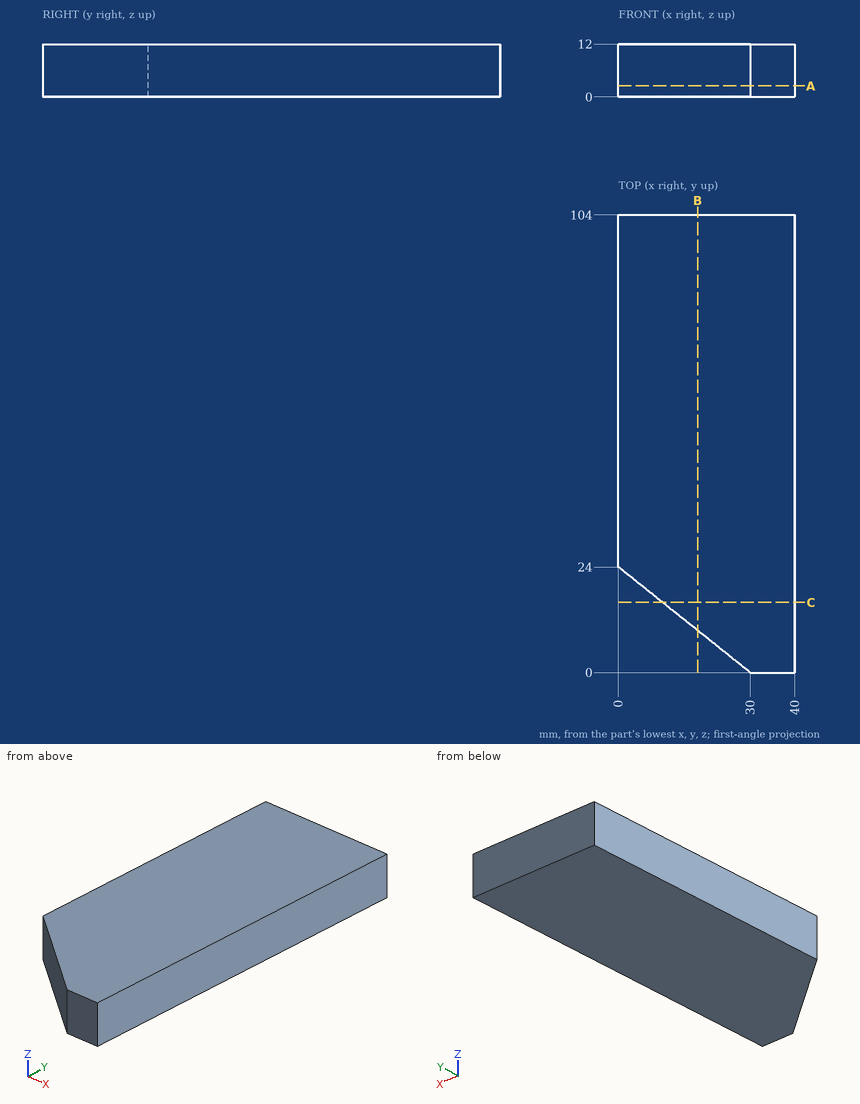
The drawing under review shows one solid part. Ordinate dimensions are in mm from its lowest x, y, z. Round coordinates to 2 decimals unless told otherwise and drop trailing zeros. Write each loop counter-clockwise with the first axis right and the second up, starting at its lowest first coordinate (ties: lowest second). Pieces come first, ordered by that corner, then holes.
(1) We need section C-C on y = 16. Give the boundary of the cut face in (x, z), and give its area (3 significant figures).
(2) Insertion check: pin 1 (2 mm diameter, centred on y = 19, z = 5.5, fed in from -X); pin 2 (2 mm diameter, centred on x = 9.5, z = 7.5, fed in from -Y); pin 3 (6 mm diameter, centred on x = 9, z = 1.5, fed in from -Y). Each pin has a flat end and moves straight along its axis. Give the tip position at first contact, or say it passes through.
(3) We need section A-A on z = 2.5. Give the boundary of the cut face in (x, y), and give its area (3 significant figures).
(4) We need section B-B on x = 18. Give the boundary of the cut face in (y, z).
(5) Wall thickness on L1, parallel to X at y = 12, z = 3; L2, parallel to Y at x = 29, z = 1.25; L3, parallel to Y at x = 27, z = 10.5: over which ranges is each line inside the solid? List them lowest first.
Findings below:
1. outline: (10, 0) - (40, 0) - (40, 12) - (10, 12) - close
1. area: 360 mm2
2. pin 1: stops at x = 5
2. pin 2: stops at y = 15.6
2. pin 3: stops at y = 14.4
3. outline: (0, 24) - (30, 0) - (40, 0) - (40, 104) - (0, 104) - close
3. area: 3,800 mm2
4. outline: (9.6, 0) - (104, 0) - (104, 12) - (9.6, 12) - close
5. L1: x = 15 to 40
5. L2: y = 0.8 to 104
5. L3: y = 2.4 to 104
